Check sheet for the modelled part. Datum: model origin and axes. Units: mm. A direction names the side the tool comes from. Round coordinates to 2 decimals unless told otherwise and drop trailing zeros. One line per item, written item: value. Start each with the question number.
1. Go/stop test with flat-tipped pins: pin 1 (2 mm diameter, centred on y = -2, z = -2.5, fed in from +X); pin 2 (1.1 mm diameter, centred on x = -14.5, y = 0.5, fed in from +Z); pin 3 (1.8 mm diameter, centred on x = -14, y = 0, fed in from -Z). Record where each tip stops, or that it passes through.
2. Set-up check for faces 5 (the face through (-12, 3.4, 0.1)), 6 (the face through (-15.26, -1.87, -1.06)), 7 (the face through (-15.3, 2, 2)): record each of +Z, -Z, +X, -X, +Y, -Y from which the full face is reachable in a straight line by a thin tool's end or side.
3. Material ranges on L1, parallel to Z at x = -10.25, y = -0.75; L2, parallel to Y at x = -10, z = -1.75; L3, parallel to Z at x = -5.25, y = -0.5, recorded low to high.
4. Release check for a two-part mould opening along Y. For faces 1 (the face through (-6.2, -0.9, 2.86)), 2 (the face through (-14.19, -1.74, 0.99)), 3 (the face through (0, 0, 0)), 4 (the face through (-15.26, 1.87, 1.06)) record: +Y half, -Y half, draft (parallel to the pull), parting line (faces both ways), or undercut.
from build123d import *

# Parameters (mm, degrees)
CUT_EXTRUDE1_DEPTH = 3.3


with BuildPart() as part:
    # Sketch1 → Revolve1 (revolve)
    with BuildSketch(Plane.XY, mode=Mode.PRIVATE) as revolve1_sk:
        with BuildLine():
            Line((0, 3), (-11.75, 3))
            ThreePointArc((-11.75, 3), (-11.926776695, 3.073223305), (-12, 3.25))
            Line((-12, 3.25), (-12, 5.25))
            ThreePointArc((-12, 5.25), (-13.866655204, 4.442760966), (-15.3, 3))
            Line((-15.3, 3), (-15.3, 0))
            Line((-15.3, 0), (0, 0))
            Line((0, 0), (0, 3))
        make_face()
    revolve(revolve1_sk.sketch.rotate(Axis((-15.3, 0, 0), (1, 0, 0)), 90), axis=Axis((-15.3, 0, 0), (1, 0, 0)))

    # Sketch2 → Cut-Extrude1 (cut)
    with BuildSketch(Plane.ZY.offset(15.3)):
        Polygon((0, 2.309401077), (-2, 1.154700538), (-2, -1.154700538), (0, -2.309401077), (2, -1.154700538), (2, 1.154700538), align=None)
    extrude(amount=-CUT_EXTRUDE1_DEPTH, mode=Mode.SUBTRACT)

    # Sketch6 → Revolve2 (revolve)
    with BuildSketch(Plane.XY):
        Polygon((-13.22, 2.309401077), (-12, 0), (-11.42, 0), (-11.42, 2.309401077), align=None)
    revolve(axis=Axis((-15.3, 0, 0), (1, 0, 0)))

    # Sketch7 → Cut-Revolve5 (revolve, cut)
    with BuildSketch(Plane.XY):
        Polygon((-15.3, 2.309401077), (-14.72, 0), (-15.3, 0), align=None)
    revolve(axis=Axis((-15.3, 0, 0), (1, 0, 0)), mode=Mode.SUBTRACT)

    # Sketch4 → Cut-Revolve1 (revolve, cut)
    with BuildSketch(Plane.XY, mode=Mode.PRIVATE) as cut_revolve1_sk:
        Polygon((-0.5, 3), (0, 2.133974596), (0.5, 3), align=None)
    revolve(cut_revolve1_sk.sketch.rotate(Axis((-0.5, 0, 0), (1, 0, 0)), 90), axis=Axis((-0.5, 0, 0), (1, 0, 0)), mode=Mode.SUBTRACT)


solid = part.part
Taken from the geometry:
1. pin 1: stops at x = -0.04
1. pin 2: stops at z = 4.36
1. pin 3: stops at z = -4.88
2. face 5: +X
2. face 6: -X
2. face 7: +Z, -Z, -X, +Y, -Y
3. L1: z = -2.9 to 2.9
3. L2: y = -2.44 to 2.44
3. L3: z = -2.96 to 2.96
4. face 1: parting line
4. face 2: undercut
4. face 3: draft
4. face 4: undercut
